Input: part model. Units: mm. Frame: model coordinates. Face numbers are marked on the shaded views. Give positions to 0.01 mm unless a question says otherwise; leave off trailing zeros. Loops run counter-clockwise (first coordinate to the right, second up) from the corner with the lowest first, then second, coordinate; pieces in that order, holes last.
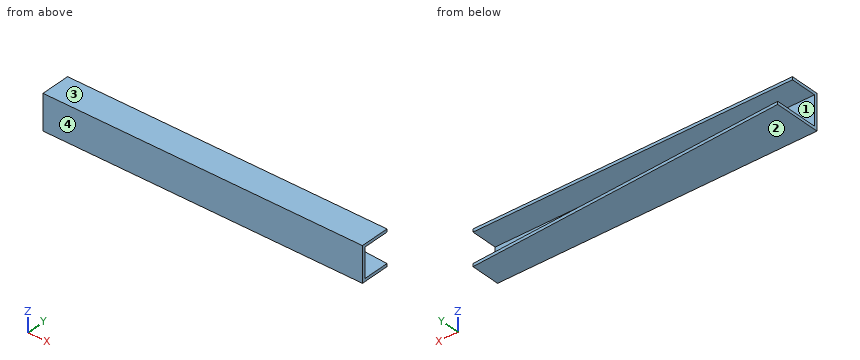
from build123d import *

# Parameters (mm, degrees)
EXTRUDE_1_DEPTH     = 60
SHELL_2_T           = -5
CUT_EXTRUDE_2_DEPTH = 38


with BuildPart() as part:
    # 草图1 → 凸台-拉伸1 (new body)
    with BuildSketch(Plane.XY):
        Polygon((0, 0), (0, -80), (545, -80), (545, -30), align=None)
    extrude(amount=EXTRUDE_1_DEPTH)

    # 抽壳2
    shell_2_openings = [part.faces().sort_by_distance(p)[0] for p in [
        (545, -55, 30),
        (0, -40, 30),
        (272.5, -15, 30),
    ]]
    offset(amount=SHELL_2_T, openings=shell_2_openings, kind=Kind.INTERSECTION)

    # 草图4 → 切除-拉伸2 (cut)
    with BuildSketch(Plane.XY.offset(60)):
        Polygon((545, -30), (0, -30), (0, 50.034428037), align=None)
    extrude(amount=-CUT_EXTRUDE_2_DEPTH, mode=Mode.SUBTRACT)


solid = part.part
(1) Pin query (flat end, axial travel): pin 1 Ø4 at (x, z) = (366.5, 9.5) entering from +Y; pin 2 Ø8 at (y, z) = (-43, 50) entering from -X; pin 3 Ø1.5 at (x, z) = (180.5, 57) entering from +Y. Return the tip coordinate at first contact, or that it passes through.
Values follow:
pin 1: stops at y = -75
pin 2: passes through
pin 3: stops at y = -30
(2) Mould query, pull axis Z, two halves, no side actions, for the marked faces 1, 2, 3 and 4. Classes: +Z half, -Z half, draft (parallel to the pull), parting line (faces both ways), or undercut.
Values follow:
face 1: undercut
face 2: -Z half
face 3: +Z half
face 4: draft
(3) Ray query, probe 1 along Z at (x, y) = (58, -62); probe 2 along Y at (x, z) = (212, 24); probe 3 along Y at (x, z) = (120.5, 57). Return the intervals inside material, ascending.
Values follow:
probe 1: z = 0 to 5, 55 to 60
probe 2: y = -80 to -75
probe 3: y = -80 to -30
(4) Cut plane A-A (y = -42). Return the cut outline in (x, z).
Values follow:
outline: (0, 0) - (545, 0) - (545, 5) - (0, 5) - close; (0, 55) - (545, 55) - (545, 60) - (0, 60) - close
(5) Cut plane D-D (y = -8.5). Return the cut outline in (x, z), and give its area (3 significant figures).
Values follow:
outline: (0, 0) - (154.42, 0) - (154.42, 5) - (0, 5) - close
area: 772 mm2
(6) Cut plane B-B (x = 350). Return the cut outline in (y, z).
Values follow:
outline: (-80, 0) - (-19.27, 0) - (-19.27, 5) - (-75, 5) - (-75, 55) - (-30, 55) - (-30, 60) - (-80, 60) - close
(7) Cut plane C-C (z = 28). Return the cut outline in (x, y), and give its area (4 significant figures).
Values follow:
outline: (0, -80) - (545, -80) - (545, -75) - (0, -75) - close
area: 2,725 mm2
